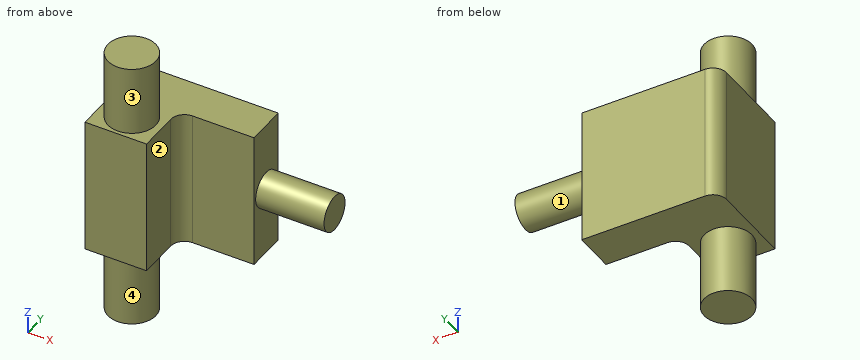
from build123d import *

# Parameters (mm, degrees)
SKETCH1_W           = 100
SKETCH1_H           = 100
BOSS_EXTRUDE1_DEPTH = 70
SKETCH2_W           = 55
SKETCH2_H           = 40
CUT_EXTRUDE1_DEPTH  = 137.037678604
SKETCH3_W           = 50
SKETCH3_H           = 13
SKETCH4_W           = 17.5
SKETCH4_H           = 50.435
SKETCH5_W           = 17.5
SKETCH5_H           = 50.435
FILLET1_R           = 10


with BuildPart() as part:
    # Sketch1 → Boss-Extrude1 (new body)
    with BuildSketch(Plane.XZ.offset(20)):
        with Locations((27.5, 0)):
            Rectangle(SKETCH1_W, SKETCH1_H)
    extrude(amount=-BOSS_EXTRUDE1_DEPTH)

    # Sketch2 → Cut-Extrude1 (cut, through all)
    with BuildSketch(Plane(origin=(0, 0, -50), x_dir=(-1, 0, 0), z_dir=(0, 0, -1))):
        with Locations((-50, 0)):
            Rectangle(SKETCH2_W, SKETCH2_H)
    extrude(amount=-CUT_EXTRUDE1_DEPTH, mode=Mode.SUBTRACT)

    # Sketch3 → Revolve1 (revolve)
    with BuildSketch(Plane(origin=(0, 0, 0), x_dir=(-1, 0, 0), z_dir=(0, 0, -1)), mode=Mode.PRIVATE) as revolve1_sk:
        with Locations((-102.5, 41.5)):
            Rectangle(SKETCH3_W, SKETCH3_H)
    revolve(revolve1_sk.sketch.rotate(Axis((127.5, 35, 0), (-1, 0, 0)), 270), axis=Axis((127.5, 35, 0), (-1, 0, 0)))

    # Sketch4 → Revolve2 (revolve)
    with BuildSketch(Plane.XZ, mode=Mode.PRIVATE) as revolve2_sk:
        with Locations((8.75, -75.2175)):
            Rectangle(SKETCH4_W, SKETCH4_H)
    revolve(revolve2_sk.sketch.rotate(Axis((0, 0, -50), (0, 0, -1)), 180), axis=Axis((0, 0, -50), (0, 0, -1)))

    # Sketch5 → Revolve3 (revolve)
    with BuildSketch(Plane.XZ, mode=Mode.PRIVATE) as revolve3_sk:
        with Locations((8.75, 75.2175)):
            Rectangle(SKETCH5_W, SKETCH5_H)
    revolve(revolve3_sk.sketch.rotate(Axis((0, 0, 100.435), (0, 0, -1)), 180), axis=Axis((0, 0, 100.435), (0, 0, -1)))

    # Fillet1
    fillet1_edges = [part.edges().sort_by_distance(p)[0] for p in [
        (22.5, 20, 0),
        (-22.5, 50, 0),
    ]]
    fillet(fillet1_edges, radius=FILLET1_R)


solid = part.part
Could you check a few things on this model? Use its own coordinates, in mm. Face numbers are marked on the shaded views. A direction names the side the tool comes from. Round coordinates to 2 decimals unless told otherwise and drop trailing zeros. Write each loop counter-clockwise with the first axis right and the second up, starting at its lowest first coordinate (ties: lowest second). Pieces come first, ordered by that corner, then holes. Notation, with made-up numbers: (-31, 54.25) - (17, 54.25) arc R21 ccw to (17, 72.25) - close; hole circle Ø6 at (-36.75, 16.25). An arc over 180 degrees is marked (long way). Put each result on its own line as item: value. Start each with the question number.
(1) Will these pins go through, and if not, where does the flat tip stop? pin 1 (5 mm diameter, centred on x = 73.5, y = 23, fed in from -Z); pin 2 (8 mm diameter, centred on y = 31, z = -53, fed in from +X); pin 3 (4 mm diameter, centred on y = 6.5, z = -79.5, fed in from +X).
(2) I need wall thicknesses on probe 1 along X at (y, z) = (-12, 9); probe 2 along Z at (x, y) = (19, 23.5); probe 3 along X at (y, z) = (32.5, -33). Which ranges of each line are inside material? Lowest first, please.
(3) I want a section at A-A, the plane x = 0. Please give me the cut outline in (y, z) (3 decimals).
(4) I want a section at B-B, the plane z = 0. Please give me the cut outline in (x, y), plus the area to 3 significant figures.
(5) I want a section at D-D, the plane z = -30. Please give me the cut outline in (x, y), plus the area to 3 significant figures.
(6) For the marked faces 1, 2, 3 and 4, which set-ups out of +Z, -Z, +X, -X, +Y, -Y let a thin tool reach every point of the face, with its end or its side?
(7) I want a section at C-C, the plane y = 35. Please give me the cut outline in (x, z), plus the area to 3 significant figures.
Here are the results:
1. pin 1: stops at z = -50
1. pin 2: stops at x = 77.5
1. pin 3: stops at x = 16.91
2. probe 1: x = -22.5 to 22.5
2. probe 2: z = -50 to 50
2. probe 3: x = -22.5 to 77.5
3. outline: (-20, -50) - (-17.5, -50) - (-17.5, -100.435) - (17.5, -100.435) - (17.5, -50) - (50, -50) - (50, 50) - (17.5, 50) - (17.5, 100.435) - (-17.5, 100.435) - (-17.5, 50) - (-20, 50) - close
4. outline: (-22.5, -20) - (22.5, -20) - (22.5, 10) arc R10 cw to (32.5, 20) - (77.5, 20) - (77.5, 22) - (127.5, 22) - (127.5, 48) - (77.5, 48) - (77.5, 50) - (-12.5, 50) arc R10 ccw to (-22.5, 40) - close
4. area: 6,100 mm^2
5. outline: (-22.5, -20) - (22.5, -20) - (22.5, 10) arc R10 cw to (32.5, 20) - (77.5, 20) - (77.5, 50) - (-12.5, 50) arc R10 ccw to (-22.5, 40) - close
5. area: 4,800 mm^2
6. face 1: +X
6. face 2: +Z, -Z, +X, -Y
6. face 3: +Z
6. face 4: -Z
7. outline: (-22.5, -50) - (77.5, -50) - (77.5, -13) - (127.5, -13) - (127.5, 13) - (77.5, 13) - (77.5, 50) - (-22.5, 50) - close
7. area: 11,300 mm^2
